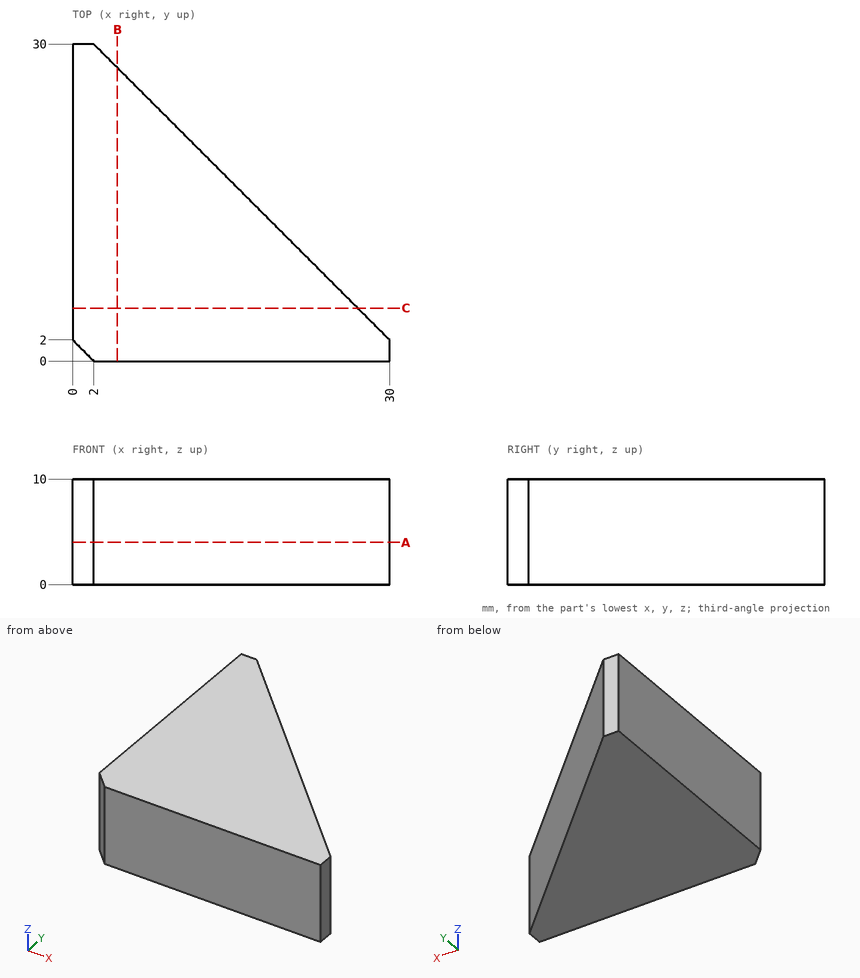
For this review, use the dimensioned drawing (mm, ordinates from the lowest corner) and the shaded views. Round coordinates to 2 decimals unless told otherwise and drop trailing zeros. Write each loop counter-clockwise with the first axis right and the second up, starting at its lowest first coordinate (ties: lowest second). Pieces come first, ordered by that corner, then holes. Notation, with made-up numbers: M 31.5,69 L 38.5,69 A23 cw 38.5,78 Z; hole C 32,24.25 d10. An arc over 180 degrees is marked long. Use CSV: the item, a comma, the result in double quotes. Start each with the question number.
(1) We need section A-A, the plane z = 4. State the section outline as (x, y) points, then the cut area to 3 significant figures.
(2) For line 1 along X through (y, z) = (7, 7); line 2 along Y through (x, z) = (13, 4); line 3 along X through (y, z) = (21.5, 2.75), list the stretches that pass through material, from the lowest coordinate up.
(3) Clearance check with flat-ended pins moving along their axes: P1, Ø2, axis at x = 6, y = 13, coming from the -Z side; P2, Ø4, axis at x = 17, z = 3.5, coming from the +Y side; P3, Ø6, axis at x = 24.5, y = 15.5, coming from the +Z side. State where each tip first meets the part, or that it passes through.
(4) We need section C-C, the plane y = 5. State the section outline as (x, z) points, then the cut area to 3 significant figures.
(5) We need section B-B, the plane x = 4.25. State the section outline as (y, z) points, then the cut area to 4 significant figures.
Findings:
1,outline,"M 0,2 L 2,0 L 30,0 L 30,2 L 2,30 L 0,30 Z"
1,area,"506 mm^2"
2,line 1,"0 to 25"
2,line 2,"0 to 19"
2,line 3,"0 to 10.5"
3,P1,"z = 0"
3,P2,"y = 17"
3,P3,"through"
4,outline,"M 0,0 L 27,0 L 27,10 L 0,10 Z"
4,area,"270 mm^2"
5,outline,"M 0,0 L 27.75,0 L 27.75,10 L 0,10 Z"
5,area,"277.5 mm^2"
